Geometry: final body of the model. Coordinates: model frame, mm. Round coordinates to 2 decimals unless told otherwise and drop trailing zeros. Loops run counter-clockwise (first coordinate to the right, second up) from the corner with the lowest first, then second, coordinate; pieces in that order, holes last. Notation, with made-up numbers: (-36.5, 41) - (-28.5, 41) arc R21 ccw to (-28.5, 79) - close; hole circle Ø6 at (-30.75, 26). An arc over 180 degrees is marked (long way). Return JSON: item names as keys, results as strings. Group by question number.
1. Section A-A on z = 8.5. Return loops of the section in (x, y).
2. Section B-B on y = 40. Return loops of the section in (x, z).
3. Section C-C on x = 100. Return loops of the section in (y, z).
4. Material intervals for probe 1 along Y at (x, z) = (-100, 19); probe 2 along X at (y, z) = (33, 34); probe 3 along X at (y, z) = (45, 14), sorted ascending.
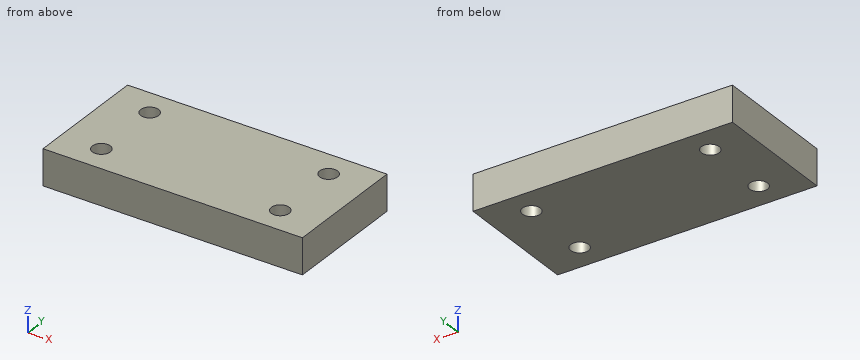
from build123d import *

# Parameters (mm, degrees)
SKETCH1_W           = 290
SKETCH1_H           = 140
SKETCH1_R           = 10
BOSS_EXTRUDE1_DEPTH = 40


with BuildPart() as part:
    # Sketch1 → Boss-Extrude1 (new body)
    with BuildSketch(Plane.XY):
        Rectangle(SKETCH1_W, SKETCH1_H)
        with Locations((-100, 40)):
            Circle(SKETCH1_R, mode=Mode.SUBTRACT)
        with Locations((-100, -40)):
            Circle(SKETCH1_R, mode=Mode.SUBTRACT)
        with Locations(Location((100, -40, 0), (0, 0, 180))):
            Circle(SKETCH1_R, mode=Mode.SUBTRACT)
        with Locations(Location((100, 40, 0), (0, 0, 180))):
            Circle(SKETCH1_R, mode=Mode.SUBTRACT)
    extrude(amount=BOSS_EXTRUDE1_DEPTH)


solid = part.part
Taken from the geometry:
{
 "1": {"outline": "(-145, -70) - (145, -70) - (145, 70) - (-145, 70) - close; hole circle Ø20 at (-100, -40); hole circle Ø20 at (-100, 40); hole circle Ø20 at (100, -40); hole circle Ø20 at (100, 40)"},
 "2": {"outline": "(-145, 0) - (-110, 0) - (-110, 40) - (-145, 40) - close; (-90, 0) - (90, 0) - (90, 40) - (-90, 40) - close; (110, 0) - (145, 0) - (145, 40) - (110, 40) - close"},
 "3": {"outline": "(-70, 0) - (-50, 0) - (-50, 40) - (-70, 40) - close; (-30, 0) - (30, 0) - (30, 40) - (-30, 40) - close; (50, 0) - (70, 0) - (70, 40) - (50, 40) - close"},
 "4": {"probe 1": "-70 to -50, -30 to 30, 50 to 70", "probe 2": "-145 to -107.14, -92.86 to 92.86, 107.14 to 145", "probe 3": "-145 to -108.66, -91.34 to 91.34, 108.66 to 145"}
}
